CAD build for the part. Positions are in the model's coordinates, mm. Give positions to 0.01 mm unless a question says otherwise; leave off trailing zeros. Order: outer loops, then holes, each group sorted by start corner. A loop starts at its lowest first (then second) coordinate and runs counter-clockwise, first axis right, second up.
```python
from build123d import *

# Parameters (mm, degrees)
SKETCH_1_R      = 2.5
EXTRUDE_1_DEPTH = 3
FILLET_1_R      = 10


with BuildPart() as part:
    # 草图1 → 凸台-拉伸1 (new body)
    with BuildSketch(Plane(origin=(0, 0, 0), x_dir=(1, 0, 0), z_dir=(0, 1, 0))):
        with BuildLine():
            Line((3, -4), (47, -4))
            ThreePointArc((47, -4), (55, 0), (47, 4))
            Line((47, 4), (3, 4))
            ThreePointArc((3, 4), (-5, 0), (3, -4))
        make_face()
        with Locations(Location((0, 0, 0), (0, 0, 270))):
            Circle(SKETCH_1_R, mode=Mode.SUBTRACT)
        with Locations(Location((50, 0, 0), (0, 0, 270))):
            Circle(SKETCH_1_R, mode=Mode.SUBTRACT)
    extrude(amount=EXTRUDE_1_DEPTH)

    # 圆角1
    fillet_1_edges = [part.edges().sort_by_distance(p)[0] for p in [
        (3, 1.5, -4),
        (47, 1.5, -4),
        (47, 1.5, 4),
        (3, 1.5, 4),
    ]]
    fillet(fillet_1_edges, radius=FILLET_1_R)


solid = part.part
```
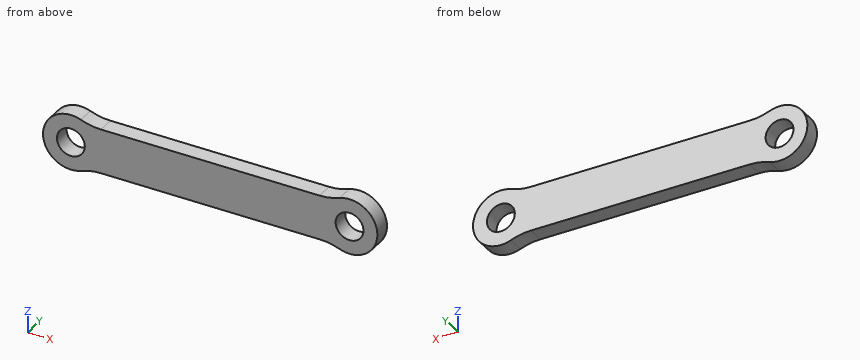
Item 1: Drop flat-ended pins along their axis: pin 1 Ø1 at (x, y) = (16, 2.5) entering from +Z; pin 2 Ø6 at (x, z) = (50, 0) entering from -Y; pin 3 Ø1.5 at (x, y) = (32.5, 1.5) entering from -Z. Give the stop position or say it passes through.
Item 2: Slice it at A-A (x = 50). Give the cut face in (y, z).
Item 3: Slice it at D-D (x = 1). Give the cut face in (y, z), and give its area (3 significant figures).
Item 4: Wall check: L1, parallel to X at y = 2.1, z = -2; L2, parallel to X at y = 0.6, z = -1.5; L3, parallel to Z at x = 38, y = 0.55. Give the ranges that are in metal, low to high.
Item 5: Slice it at C-C (y = 1). Give the cut face in (x, z), and give its area (3 significant figures).
Item 6: Slice it at B-B (z = 0). Give the cut face in (x, y).
A:
1. pin 1: stops at z = 4
1. pin 2: stops at y = 0
1. pin 3: stops at z = -4
2. outline: (0, -5) - (3, -5) - (3, -2.5) - (0, -2.5) - close; (0, 2.5) - (3, 2.5) - (3, 5) - (0, 5) - close
3. outline: (0, -4.9) - (3, -4.9) - (3, -2.29) - (0, -2.29) - close; (0, 2.29) - (3, 2.29) - (3, 4.9) - (0, 4.9) - close
3. area: 15.6 mm2
4. L1: x = -4.58 to -1.5, 1.5 to 48.5, 51.5 to 54.58
4. L2: x = -4.77 to -2, 2 to 48, 52 to 54.77
4. L3: z = -4 to 4
5. outline: (1.8, -4.67) arc R10 cw to (5.39, -4) - (44.61, -4) arc R10 cw to (48.2, -4.67) arc R5 ccw (long way) to (48.2, 4.67) arc R10 cw to (44.61, 4) - (5.39, 4) arc R10 cw to (1.8, 4.67) arc R5 ccw (long way) to start; hole circle Ø5 at (0, 0); hole circle Ø5 at (50, 0)
5. area: 449 mm2
6. outline: (-5, 0) - (-2.5, 0) - (-2.5, 3) - (-5, 3) - close; (2.5, 0) - (47.5, 0) - (47.5, 3) - (2.5, 3) - close; (52.5, 0) - (55, 0) - (55, 3) - (52.5, 3) - close
